Model file for the job. Use its own axes, mm. Face numbers are marked on the shaded views. A direction names the side the tool comes from. Coordinates: 2 decimals unless noted, no trailing zeros. Loops run counter-clockwise (first coordinate to the right, second up) from the corner with the lowest first, then second, coordinate; pieces in that order, holes last. Notation, with made-up numbers: (-27, 39.25) -> (-22, 39.25) arc R22 ccw to (-22, 57.25) -> close; hole circle Ø6 at (-19.5, 2.5). An arc over 180 degrees is marked (long way). Use one line per item in the form item = value.
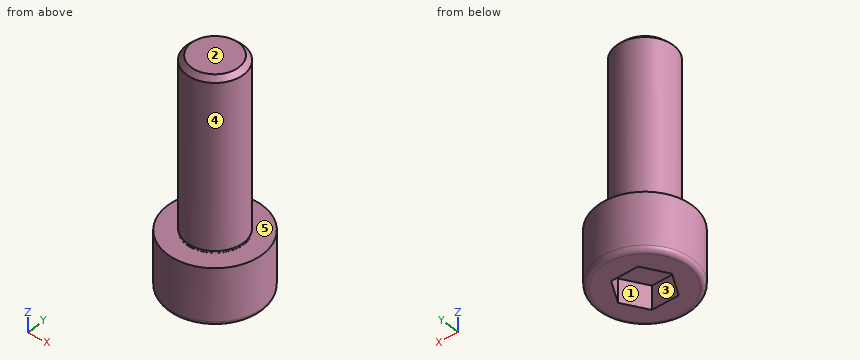
```python
from build123d import *

# Parameters (mm, degrees)
CUT_EXTRUDE1_DEPTH = 2.5


with BuildPart() as part:
    # Logo3_bib1 → Revolve1 (revolve)
    with BuildSketch(Plane(origin=(0, 0, 0), x_dir=(-1, 0, 0), z_dir=(0, -1, 0))):
        with BuildLine():
            Line((0, -18), (0, 6))
            Line((0, 6), (4.5, 6))
            ThreePointArc((4.5, 6), (4.853553391, 5.853553391), (5, 5.5))
            Line((5, 5.5), (5, 0))
            Line((5, 0), (3, 0))
            Line((3, 0), (3, -0.01))
            Line((3, -0.01), (2.613425636, -0.01))
            ThreePointArc((2.613425636, -0.01), (2.593729481, -0.026527036), (2.606585234, -0.048793852))
            Line((2.606585234, -0.048793852), (3, -0.191985117))
            Line((3, -0.191985117), (3, -17.5))
            Line((3, -17.5), (2.5, -18))
            Line((2.5, -18), (0, -18))
        make_face()
    revolve(axis=Axis((0, 0, -10.585154653), (0, 0, 1)))

    # Logo3_bib2 → Cut-Extrude1 (cut)
    with BuildSketch(Plane(origin=(0, 0, -6), x_dir=(1, 0, 0), z_dir=(0, 0, -1))):
        Polygon((2.886751346, 0), (1.443375673, 2.5), (-1.443375673, 2.5), (-2.886751346, 0), (-1.443375673, -2.5), (1.443375673, -2.5), align=None)
    extrude(amount=-CUT_EXTRUDE1_DEPTH, mode=Mode.SUBTRACT)


solid = part.part
```
Q1. Band-saw the part on A-A, the plane z = -4. Write the cut outline in (x, y).
Result:
outline = circle Ø10 at (0, 0); hole (-2.89, 0) -> (-1.44, -2.5) -> (1.44, -2.5) -> (2.89, 0) -> (1.44, 2.5) -> (-1.44, 2.5) -> close
Q2. Pin check, flat tips, straight feed: pin 1 Ø1.5 at (x, y) = (0, -3.5) entering from +Z; pin 2 Ø4 at (y, z) = (1.5, 10.5) entering from +X; pin 3 Ø1.5 at (x, y) = (-1, 0.5) entering from -Z. Stop position of each tip, or through.
Result:
pin_1 = 17.75
pin_2 = 3
pin_3 = -3.5
Q3. Which spindle directions (+Z, -Z, +X, -X, +Y, -Y) get a long thin tool onto all of the face, cutting with end or side? Do the marked faces 1 and 2. Say none if no direction does.
Result:
face_1 = -Z
face_2 = +Z, +X, -X, +Y, -Y
Q4. Band-saw the part on C-C, the plane z = 10. Write the cut outline in (x, y).
Result:
outline = circle Ø6 at (0, 0)
Q5. Wall check: line 1 along Y through (x, z) = (0, -4.5); line 2 along Z through (x, y) = (-1.5, 0); line 3 along Z through (x, y) = (0.25, 3.25). Give the ranges that are in metal, low to high.
Result:
line_1 = -5 to -2.5, 2.5 to 5
line_2 = -3.5 to 18
line_3 = -6 to 0
Q6. Mould opens along Y. For the marked faces 3, 4 and 5 say: released by +Y, released by -Y, zero draft, split by the parting line, or undercut.
Result:
face_3 = undercut
face_4 = split by the parting line
face_5 = zero draft
